Read the model definition and answer for the solid it produces. Units are mm, in the model's axes. Face numbers are marked on the shaded views. Give positions to 0.01 mm unless a question says otherwise; leave off trailing zeros. Loops run counter-clockwise (first coordinate to the right, second up) from the corner with the lowest first, then second, coordinate; pieces in that order, holes last. Notation, with made-up numbers: (84.5, -25) - (123.5, -25) arc R19 ccw to (123.5, -16) - close; hole circle Ø11 at (63, 75.25). An arc over 180 degrees is marked (long way). Put each result on its own line as item: value. Start each with the question number.
1. A cutting plane is placed at B-B, the plane y = 32.5. Determine the outline of the cut face in (x, z).
2. A cutting plane is placed at D-D, the plane x = 60. Determine the outline of the cut face in (y, z), plus the area to 3 significant figures.
3. Given pin 1 Ø3 at (x, z) = (30.5, 4) entering from -Y; pin 2 Ø3 at (x, z) = (14, 5) entering from +Y, each flat-ended and moving along its own axis, determine where each tip first touches the part or whether it passes through.
4. For a pull along X with two mould halves and no side action, classify the marked faces 1, 2, 3 and 4 as released by +X, released by -X, zero draft, split by the parting line, or undercut.
5. A cutting plane is placed at C-C, the plane x = 35. Determine the outline of the cut face in (y, z), plus the area to 3 significant figures.
6. A cutting plane is placed at A-A, the plane z = 4.75. Determine the outline of the cut face in (x, y), plus the area to 3 significant figures.
7. Consider L1, parallel to Y at x = 35, z = 4.7; L2, parallel to X at y = 33.5, z = 1.9; L3, parallel to Y at x = 30, z = 2.6. Determine where each line is inside the solid, lowest interval first. Write a range as from..to.
```python
from build123d import *

# Parameters (mm, degrees)
BOSS_EXTRUDE1_DEPTH    = 6
M10_TAPPED_HOLE2_D     = 8.5
M10_TAPPED_HOLE2_DEPTH = 24.5
M10_TAPPED_HOLE2_TIP   = 2.553657631
CHAMFER1_SIZE          = 4
CHAMFER1_SIZE2         = 4.024049749


with BuildPart() as part:
    # Sketch1 → Boss-Extrude1 (new body)
    with BuildSketch(Plane.XY):
        Polygon((0, 0), (0, 60), (68.372865684, 50.718230869), (64, 17), (10, 0), align=None)
    extrude(amount=BOSS_EXTRUDE1_DEPTH)

    # M10 Tapped Hole2
    with Locations(Plane.XY.offset(6)):
        with Locations((35, 30)):
            Hole(M10_TAPPED_HOLE2_D / 2, depth=M10_TAPPED_HOLE2_DEPTH)
            with Locations((0, 0, -(M10_TAPPED_HOLE2_DEPTH + M10_TAPPED_HOLE2_TIP / 2))):  # 118° drill point
                Cone(0, M10_TAPPED_HOLE2_D / 2, M10_TAPPED_HOLE2_TIP, mode=Mode.SUBTRACT)

    # Chamfer1
    chamfer1_edges = [part.edges().sort_by_distance(p)[0] for p in [
        (68.372865684, 50.718230869, 3),
    ]]
    chamfer1_side = [part.faces().sort_by_distance(p)[0] for p in [
        (66.186432842, 33.859115434, 3),
    ]]
    chamfer(chamfer1_edges, length=CHAMFER1_SIZE, length2=CHAMFER1_SIZE2, reference=chamfer1_side[0])


solid = part.part
```
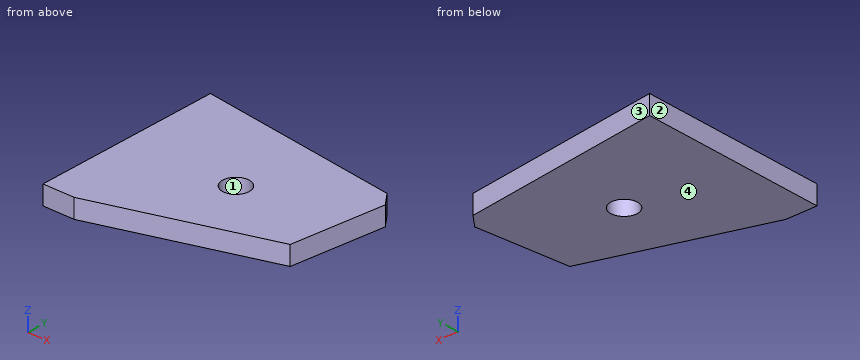
Return value:
1. outline: (0, 0) - (31.56, 0) - (31.56, 6) - (0, 6) - close; (38.44, 0) - (66.01, 0) - (66.01, 6) - (38.44, 6) - close
2. outline: (15.74, 0) - (51.85, 0) - (51.85, 6) - (15.74, 6) - close
2. area: 217 mm2
3. pin 1: stops at y = 5.98
3. pin 2: stops at y = 58.3
4. face 1: undercut
4. face 2: released by -X
4. face 3: released by +X
4. face 4: zero draft
5. outline: (7.87, 0) - (25.75, 0) - (25.75, 6) - (7.87, 6) - close; (34.25, 0) - (55.25, 0) - (55.25, 6) - (34.25, 6) - close
5. area: 233 mm2
6. outline: (0, 0) - (10, 0) - (64, 17) - (67.86, 46.75) - (64.39, 51.26) - (0, 60) - close; hole circle Ø8.5 at (35, 30)
6. area: 3,110 mm2
7. L1: y = 7.87..25.75, 34.25..55.25
7. L2: x = 0..32.59, 37.41..66.14
7. L3: y = 6.3..55.93
